```python
from build123d import *

# Parameters (mm, degrees)
BOSS_EXTRUDE1_DEPTH = 22.5
CHAMFER1_SIZE       = 10


with BuildPart() as part:
    # Sketch1 → Boss-Extrude1 (new, symmetric)
    with BuildSketch(Plane(origin=(0, 0, 0), x_dir=(0, 0, -1), z_dir=(1, 0, 0))):
        with BuildLine():
            Line((0, 0), (0, 180))
            ThreePointArc((0, 180), (-28.284271247, 191.715728753), (-40, 220))
            Line((-40, 220), (-140, 220))
            Line((-140, 220), (-140, 180))
            Line((-140, 180), (-40, 0))
            Line((-40, 0), (0, 0))
        make_face()
    extrude(amount=BOSS_EXTRUDE1_DEPTH, both=True)

    # Chamfer1
    chamfer1_edges = [part.edges().sort_by_distance(p)[0] for p in [
        (22.5, 220, 90),
        (-22.5, 220, 90),
        (22.5, 90, 0),
        (-22.5, 90, 0),
    ]]
    chamfer(chamfer1_edges, length=CHAMFER1_SIZE)


solid = part.part
```
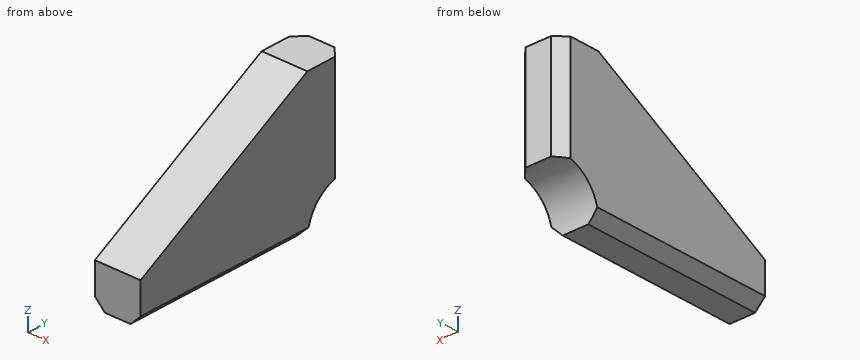
Work out the finished part from the listing and answer in its coordinate system (mm). Round coordinates to 2 decimals unless told otherwise and drop trailing zeros. Order: outer loops, then holes, each group sorted by start corner. A loop starts at its lowest first (then second) coordinate and runs counter-clockwise, first axis right, second up.
Q1. Given pin 1 Ø6 at (x, z) = (-8, 104) entering from -Y; pin 2 Ø12 at (x, y) = (-2, 27.5) entering from +Z; pin 3 Ø2 at (x, z) = (-3, 108) entering from -Y, each flat-ended and moving along its own axis, determine where each tip first touches the part or whether it passes through.
Solution:
pin 1: stops at y = 109.8
pin 2: stops at z = 58.61
pin 3: stops at y = 120.6
Q2. A cutting plane is placed at B-B, the plane y = 148.5. Determine the outline of the cut face in (x, z), then the cut area to 3 significant figures.
Solution:
outline: (-22.5, 10) - (-12.5, 0) - (12.5, 0) - (22.5, 10) - (22.5, 122.5) - (-22.5, 122.5) - close
area: 5,410 mm2
Q3. A cutting plane is placed at C-C, the plane z = 26. Determine the outline of the cut face in (x, y), then the cut area to 3 significant figures.
Solution:
outline: (-22.5, 0) - (22.5, 0) - (22.5, 189.6) - (-22.5, 189.6) - close
area: 8,530 mm2
Q4. Find the intervals of material crossed by line 1 along Y through (x, z) = (-5, 118); line 2 along X through (y, z) = (81, 6); line 3 along Y through (x, z) = (6.5, 26.5), in increasing order.
Solution:
line 1: y = 140.4 to 220
line 2: x = -18.5 to 18.5
line 3: y = 0 to 190.04
Q5. A cutting plane is placed at A-A, the plane z = 46. Determine the outline of the cut face in (x, y), then the cut area to 3 significant figures.
Solution:
outline: (-22.5, 10.8) - (22.5, 10.8) - (22.5, 210) - (12.5, 220) - (-12.5, 220) - (-22.5, 210) - close
area: 9,310 mm2
